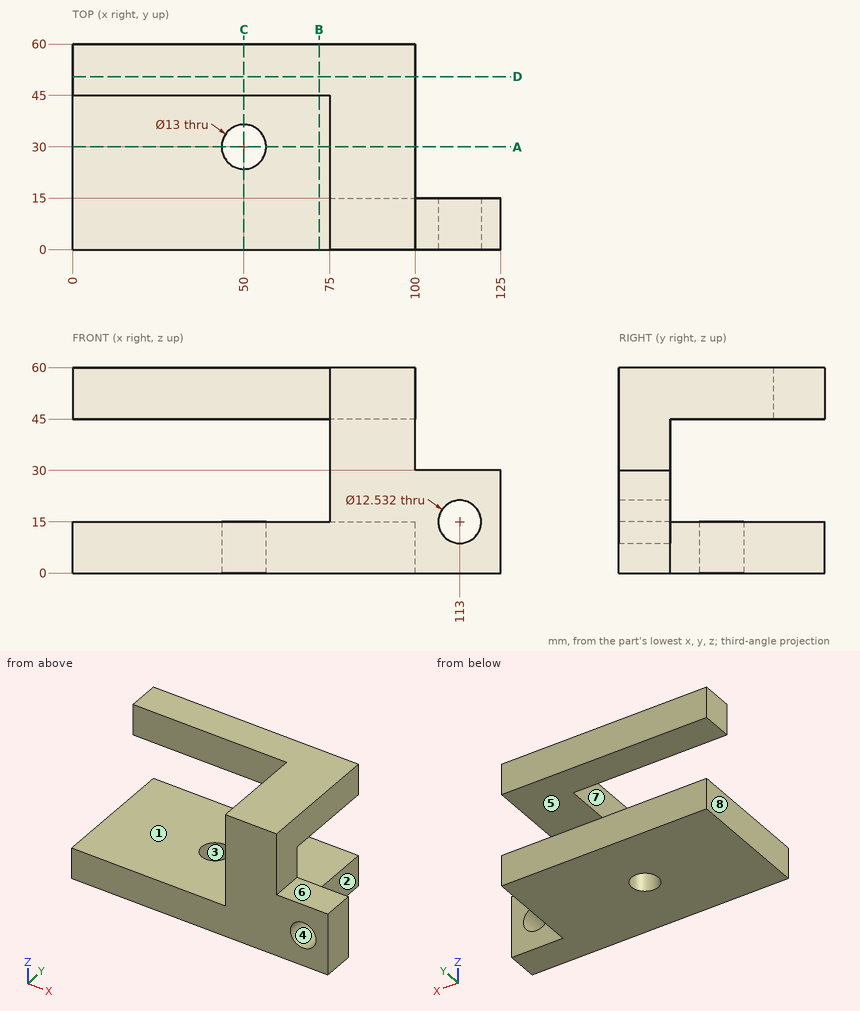
Design review of the part shown in the three views and the two pictorial views. Dimensions are in mm from the part's minimum x, y and z. A direction names the side the tool comes from. Coordinates: 2 decimals unless noted, no trailing zeros. Order: outer loops, then holes, each group sorted by start corner. A loop starts at its lowest first (then second) coordinate and runs counter-clockwise, first axis right, second up. Notation, with made-up numbers: (87, 44.25) - (125, 44.25) arc R14 cw to (125, 53.25) - close; hole circle Ø7 at (80, 13). An arc over 180 degrees is marked (long way). One line per question, with ' | ' between items.
Q1. To check wall thickness, follow line 1 along Y through (x, z) = (50, 5); line 2 along Z through (x, y) = (68.5, 50); line 3 along X through (y, z) = (48, 50). State the ranges of each line that lie inside material, in increasing order.
Answer key:
line 1: y = 0 to 23.5, 36.5 to 60 | line 2: z = 0 to 15, 45 to 60 | line 3: x = 0 to 100
Q2. Consider section B-B, the plane x = 72. Give the boundary of the cut face in (y, z).
Answer key:
outline: (0, 0) - (60, 0) - (60, 15) - (0, 15) - close; (45, 45) - (60, 45) - (60, 60) - (45, 60) - close
Q3. Consider section D-D, the plane y = 50.5. Give the boundary of the cut face in (x, z).
Answer key:
outline: (0, 0) - (100, 0) - (100, 15) - (0, 15) - close; (0, 45) - (100, 45) - (100, 60) - (0, 60) - close
Q4. The part is to be moulded in two halves that separate along X. For the marked faces 1, 2, 3 and 4, say which applies: +X half, -X half, draft (parallel to the pull), parting line (faces both ways), or undercut.
Answer key:
face 1: draft | face 2: +X half | face 3: undercut | face 4: undercut
Q5. For the marked faces 5, 6, 7 and 8, list the 3-axis set-ups (+Z, -Z, +X, -X, +Y, -Y) from which the entire face can be reached by the end or side of a thin tool; tool diameter is ignored.
Answer key:
face 5: +X, -X, +Y | face 6: +Z, +X, +Y, -Y | face 7: +Z, -X, -Y | face 8: +Z, -Z, -X, +Y, -Y
Q6. Consider section C-C, the plane x = 50. Give the boundary of the cut face in (y, z).
Answer key:
outline: (0, 0) - (23.5, 0) - (23.5, 15) - (0, 15) - close; (36.5, 0) - (60, 0) - (60, 15) - (36.5, 15) - close; (45, 45) - (60, 45) - (60, 60) - (45, 60) - close
Q7. Clearance check with flat-ended pins moving along their axes: pin 1 Ø12 at (x, y) = (57.5, 11.5) entering from -Z; pin 2 Ø4.5 at (x, z) = (39, 54.5) entering from -Y; pin 3 Ø1 at (x, z) = (13.5, 43) entering from +Y; pin 4 Ø13.5 at (y, z) = (27.5, 38.5) entering from -X. State where each tip first meets the part, or that it passes through.
Answer key:
pin 1: stops at z = 0 | pin 2: stops at y = 45 | pin 3: passes through | pin 4: stops at x = 75
Q8. Consider section A-A, the plane y = 30. Give the boundary of the cut face in (x, z).
Answer key:
outline: (0, 0) - (43.5, 0) - (43.5, 15) - (0, 15) - close; (56.5, 0) - (100, 0) - (100, 15) - (56.5, 15) - close; (75, 45) - (100, 45) - (100, 60) - (75, 60) - close
